from build123d import *

# Parameters (mm, degrees)
SKETCH_1_W                   = 68
SKETCH_1_H                   = 25
EXTRUDE_1_DEPTH              = 5
HOLE_WIZARD_M4_1_D           = 4.5
HOLE_WIZARD_M4_1_CBORE_D     = 8
HOLE_WIZARD_M4_1_CBORE_DEPTH = 4.4
CUT_EXTRUDE_1_DEPTH          = 4.4
CHAMFER_1_SIZE               = 1


with BuildPart() as part:
    # 草图1 → 凸台-拉伸1 (new, symmetric)
    with BuildSketch(Plane(origin=(0, 0, 0), x_dir=(1, 0, 0), z_dir=(0, 1, 0))):
        Rectangle(SKETCH_1_W, SKETCH_1_H)
    extrude(amount=EXTRUDE_1_DEPTH, both=True)

    # M4 六角凹头螺钉的柱形沉头孔1 (through all)
    with Locations(Plane(origin=(0, 5, 0), x_dir=(1, 0, 0), z_dir=(0, 1, 0))):
        with Locations((-28, 9), (-28, -9), (28, 9), (28, -9)):
            CounterBoreHole(HOLE_WIZARD_M4_1_D / 2, HOLE_WIZARD_M4_1_CBORE_D / 2, HOLE_WIZARD_M4_1_CBORE_DEPTH)

    # 草图4 → 切除-拉伸1 (cut)
    with BuildSketch(Plane(origin=(0, 5, 0), x_dir=(1, 0, 0), z_dir=(0, 1, 0))):
        with BuildLine():
            Line((-32, 9), (-32, 12))
            ThreePointArc((-32, 12), (-28, 16), (-24, 12))
            Line((-24, 12), (-24, 9))
            ThreePointArc((-24, 9), (-28, 5), (-32, 9))
        make_face()
        with BuildLine():
            Line((-32, -9), (-32, -12))
            ThreePointArc((-32, -12), (-28, -16), (-24, -12))
            Line((-24, -12), (-24, -9))
            ThreePointArc((-24, -9), (-28, -5), (-32, -9))
        make_face()
        with BuildLine():
            Line((32, 9), (32, 12))
            ThreePointArc((32, 12), (28, 16), (24, 12))
            Line((24, 12), (24, 9))
            ThreePointArc((24, 9), (28, 5), (32, 9))
        make_face()
        with BuildLine():
            Line((32, -9), (32, -12))
            ThreePointArc((32, -12), (28, -16), (24, -12))
            Line((24, -12), (24, -9))
            ThreePointArc((24, -9), (28, -5), (32, -9))
        make_face()
    extrude(amount=-CUT_EXTRUDE_1_DEPTH, mode=Mode.SUBTRACT)

    # 倒角1
    chamfer_1_edges = [part.edges().sort_by_distance(p)[0] for p in [
        (34, 0, 12.5),
        (-34, 0, 12.5),
        (-34, 0, -12.5),
        (34, 0, -12.5),
    ]]
    chamfer(chamfer_1_edges, length=CHAMFER_1_SIZE)


solid = part.part
CAD build for the part. Positions are in the model's coordinates, mm. Round coordinates to 2 decimals unless told otherwise and drop trailing zeros. Order: outer loops, then holes, each group sorted by start corner. A loop starts at its lowest first (then second) coordinate and runs counter-clockwise, first axis right, second up. Notation, with made-up numbers: (-2, 37) - (51, 37) arc R12 ccw to (51, 45) - close; hole circle Ø6 at (-17, -19.5). An arc over 180 degrees is marked (long way). Return JSON: item names as keys, results as strings.
(1) Pull direction X, two halves, no side cores. Call faces 1 (the face through (-29.21, -2.239, 7.103)), 2 (the face through (-34, 0, 0)), 3 (the face through (0, -5, 0)): +X half, -X half, draft (parallel to the pull), parting line (faces both ways), or undercut.
Answer key:
{"face 1": "undercut", "face 2": "-X half", "face 3": "draft"}
(2) Cut at B-B (x = 28). Give the cut face in (y, z), then the cut area to 3 significant figures.
Answer key:
{"outline": "(-5, -12.5) - (0.6, -12.5) - (0.6, -11.25) - (-5, -11.25) - close; (-5, -6.75) - (0.6, -6.75) - (0.6, -5) - (5, -5) - (5, 5) - (0.6, 5) - (0.6, 6.75) - (-5, 6.75) - close; (-5, 11.25) - (0.6, 11.25) - (0.6, 12.5) - (-5, 12.5) - close", "area": "134 mm^2"}
(3) Cut at A-A (z = 10). Give the cut face in (x, y).
Answer key:
{"outline": "(-34, -5) - (-30.02, -5) - (-30.02, 0.6) - (-32, 0.6) - (-32, 5) - (-34, 5) - close; (-25.98, -5) - (25.98, -5) - (25.98, 0.6) - (24, 0.6) - (24, 5) - (-24, 5) - (-24, 0.6) - (-25.98, 0.6) - close; (30.02, -5) - (34, -5) - (34, 5) - (32, 5) - (32, 0.6) - (30.02, 0.6) - close"}
(4) Pin check, flat tips, straight feed: pin 1 Ø4 at (x, z) = (-29.5, 8.5) entering from +Y; pin 2 Ø2 at (x, z) = (29, -9.5) entering from +Y. Stop position of each tip, or through.
Answer key:
{"pin 1": "stops at y = 0.6", "pin 2": "passes through"}
(5) Cut at D-D (z = -10.5). Give the cut face in (x, y).
Answer key:
{"outline": "(-34, -5) - (-29.68, -5) - (-29.68, 0.6) - (-32, 0.6) - (-32, 5) - (-34, 5) - close; (-26.32, -5) - (26.32, -5) - (26.32, 0.6) - (24, 0.6) - (24, 5) - (-24, 5) - (-24, 0.6) - (-26.32, 0.6) - close; (29.68, -5) - (34, -5) - (34, 5) - (32, 5) - (32, 0.6) - (29.68, 0.6) - close"}
(6) Wall check: probe 1 along Z at (x, y) = (28, -1); probe 2 along X at (y, z) = (-1, 9); probe 3 along X at (y, z) = (1.5, 10.25). Give the ranges that are in metal, low to high. Write a range as from..to.
Answer key:
{"probe 1": "z = -12.5..-11.25, -6.75..6.75, 11.25..12.5", "probe 2": "x = -34..-30.25, -25.75..25.75, 30.25..34", "probe 3": "x = -34..-32, -24..24, 32..34"}
